```python
from build123d import *

# Parameters (mm, degrees)
HEX_BODY_DEPTH                  = 65
CORNER_CHAMFER_SKETCH_OUTSIDE_W = 309.254
CORNER_CHAMFER_SKETCH_OUTSIDE_H = 330.02
CORNER_CHAMFER_SKETCH_OUTSIDE_R = 67.116968793
HEX_CORNER_CHAMFER_45DEG_DEPTH  = 65
HEX_CORNER_CHAMFER_45DEG_DRAFT  = -45
LOCKING_COLLAR_SKETCH_R         = 50
LOCKING_COLLAR_SKETCH_R_2       = 37.5
LOCKING_COLLAR_DEPTH            = 50
NUT_START                       = -120
SKETCH3_2_R                     = 37.5
NUT_BORE_DEPTH                  = 120


with BuildPart() as part:
    # Hex Profile Sketch → Hex Body (new body)
    with BuildSketch(Plane(origin=(0, 0, 0), x_dir=(1, 0, 0), z_dir=(0, 1, 0))):
        Polygon((0, -77.5), (67.116968793, -38.75), (67.116968793, 38.75), (0, 77.5), (-67.116968793, 38.75), (-67.116968793, -38.75), align=None)
    extrude(amount=HEX_BODY_DEPTH)


with BuildPart() as hex_corner_chamfer_45deg_tool:
    # Corner Chamfer Sketch outside → Hex Corner Chamfer 45deg (with draft: the straight prism first)
    with BuildSketch(Plane(origin=(0, 65, 0), x_dir=(1, 0, 0), z_dir=(0, 1, 0))):
        Rectangle(CORNER_CHAMFER_SKETCH_OUTSIDE_W, CORNER_CHAMFER_SKETCH_OUTSIDE_H)
        Circle(CORNER_CHAMFER_SKETCH_OUTSIDE_R, mode=Mode.SUBTRACT)
    extrude(amount=-HEX_CORNER_CHAMFER_45DEG_DEPTH)
    # Hex Corner Chamfer 45deg: the draft: its side faces are tilted about the plane it starts from
    hex_corner_chamfer_45deg_sides = [hex_corner_chamfer_45deg_tool.faces().sort_by_distance(p)[0] for p in [
        (0, 32.5, 165.01),
        (154.627, 32.5, 0),
        (0, 32.5, -165.01),
        (-154.627, 32.5, 0),
        (-67.116968793, 32.5, 0),
    ]]
    draft(hex_corner_chamfer_45deg_sides, Plane(origin=(0, 65, 0), x_dir=(1, 0, 0), z_dir=(0, 1, 0)), HEX_CORNER_CHAMFER_45DEG_DRAFT)


with BuildPart() as part_1:
    add(part.part)

    # Hex Corner Chamfer 45deg: cut by hex_corner_chamfer_45deg_tool
    add(hex_corner_chamfer_45deg_tool.part, mode=Mode.SUBTRACT)

    # Locking Collar Sketch → Locking Collar (add)
    with BuildSketch(Plane(origin=(0, 65, 0), x_dir=(1, 0, 0), z_dir=(0, 1, 0))):
        with Locations(Location((0, 0, 0), (0, 0, 270))):
            Circle(LOCKING_COLLAR_SKETCH_R)
        with Locations(Location((0, 0, 0), (0, 0, 270))):
            Circle(LOCKING_COLLAR_SKETCH_R_2, mode=Mode.SUBTRACT)
    extrude(amount=LOCKING_COLLAR_DEPTH)

    # Sketch3_2 → Nut Bore (cut)
    with BuildSketch(Plane(origin=(0, 65, 0), x_dir=(1, 0, 0), z_dir=(0, 1, 0)).offset(NUT_START)):
        with Locations(Location((0, 0, 0), (0, 0, 270))):
            Circle(SKETCH3_2_R)
    extrude(amount=NUT_BORE_DEPTH, mode=Mode.SUBTRACT)


solid = part_1.part
```
Input: part model. Units: mm. Frame: model coordinates. A direction names the side the tool comes from. Give positions to 0.01 mm unless a question says otherwise; leave off trailing zeros. Write each loop counter-clockwise with the first axis right and the second up, starting at its lowest first coordinate (ties: lowest second). Pieces come first, ordered by that corner, then holes. Notation, with made-up numbers: (8.5, 48) - (67.5, 48) arc R18 ccw to (67.5, 59) - close; hole circle Ø1 at (64, 54.5). An arc over 180 degrees is marked (long way). Write item = value, one per line. Start each with the question number.
1. Section query B-B, the plane y = 100.5. Output: boundary loops of the cut face in (x, z).
2. First-contact query: pin 1 Ø4 at (x, y) = (22, 91.5) entering from +Z; pin 2 Ø4 at (x, y) = (-25, 54) entering from +Z; pin 3 Ø1.5 at (x, y) = (10, 57.5) entering from +Z. Flat tips, straight axial feed; report the tip coordinate or a pass-through.
3. Mould query, pull axis Z, two halves, no side actions, for faces 1 (the flat face through (67.117, 32, 1)), 2 (the flat face through (-34.028, 32.045, 57.854)), 3 (the cylindrical face through (-22.818, 56.695, -29.759)), 4 (the conical face through (60.354, 62.525, -34.649)). Classes: released by +Z, released by -Z, zero draft, split by the parting line, or undercut.
4. Section query A-A, the plane y = 22.5. Output: boundary loops of the cut face in (x, z), then the cut area to 3 significant figures.
5. Ray query, L1, parallel to X at y = 50, z = 0; L2, parallel to X at y = 72, z = 0. Return the intervals inside material, ascending.
6. Access query for faces 5 (the flat face through (-67.117, 32, -1)), 6 (the flat face through (-50, 65, 5)). Directions: +Z, -Z, +X, -X, +Y, -Y. A direction counts if a zero-diameter tool reaches every point of the face in a straight line with its end or side. Return the directions, or none.
Check sheet entries:
q1.outline = circle Ø100 at (0, 0); hole circle Ø75 at (0, 0)
q2.pin_1 = 45.83
q2.pin_2 = 64.22
q2.pin_3 = 72.16
q3.face_1 = zero draft
q3.face_2 = released by +Z
q3.face_3 = undercut
q3.face_4 = released by -Z
q4.outline = (-67.12, -38.75) - (0, -77.5) - (67.12, -38.75) - (67.12, 38.75) - (0, 77.5) - (-67.12, 38.75) - close; hole circle Ø75 at (0, 0)
q4.area = 11,200 mm2
q5.L1 = -67.12 to -37.5, 37.5 to 67.12
q5.L2 = -50 to -37.5, 37.5 to 50
q6.face_5 = +Z, -Z, -X, +Y, -Y
q6.face_6 = +Y
